Could you check a few things on this model? Use its own coordinates, in mm. Face numbers are marked on the shaded views. A direction names the side the tool comes from. Coordinates: 2 decimals unless noted, no trailing zeros. Loops run counter-clockwise (first coordinate to the right, second up) from the corner with the lowest first, then second, coordinate; pieces in that order, holes last. Notation, with made-up numbers: (8, -23.75) - (14, -23.75) arc R11 cw to (14, -7.75) - close; hole circle Ø9 at (-31.5, -8). An arc over 180 degrees is marked (long way). Use CSV: the item, a comma, the result in double quotes.
from build123d import *

# Parameters (mm, degrees)
EXTRUDE_THIN1_DEPTH      = 10
M4_CLEARANCE_HOLE1_D     = 4.5
M4_CLEARANCE_HOLE1_DEPTH = 124.5
M4_CLEARANCE_HOLE1_TIP   = 1.351936393
FILLET1_R                = 2


with BuildPart() as part:
    # Sketch1 → Extrude-Thin1 (new body)
    with BuildSketch(Plane.XY):
        with BuildLine():
            Line((41.968719423, 0), (31.937438845, 0))
            ThreePointArc((31.937438845, 0), (15.968719423, 15), (0, 0))
            Line((0, 0), (-10.031280577, 0))
            Line((-10.031280577, 0), (-10.031280577, 2))
            Line((-10.031280577, 2), (-1.779519927, 2))
            ThreePointArc((-1.779519927, 2), (15.968719423, 17), (33.716958772, 2))
            Line((33.716958772, 2), (41.968719423, 2))
            Line((41.968719423, 2), (41.968719423, 0))
        make_face()
    extrude(amount=-EXTRUDE_THIN1_DEPTH)

    # M4 Clearance Hole1
    with Locations(Plane(origin=(0, 2, 0), x_dir=(1, 0, 0), z_dir=(0, 1, 0))):
        with Locations((-6.031280577, 5), (37.968719423, 5)):
            Hole(M4_CLEARANCE_HOLE1_D / 2, depth=M4_CLEARANCE_HOLE1_DEPTH)
            with Locations((0, 0, -(M4_CLEARANCE_HOLE1_DEPTH + M4_CLEARANCE_HOLE1_TIP / 2))):  # 118° drill point
                Cone(0, M4_CLEARANCE_HOLE1_D / 2, M4_CLEARANCE_HOLE1_TIP, mode=Mode.SUBTRACT)

    # Fillet1
    fillet1_edges = [part.edges().sort_by_distance(p)[0] for p in [
        (-10.031280577, 1, -10),
        (41.968719423, 1, -10),
        (-10.031280577, 1, 0),
        (41.968719423, 1, 0),
    ]]
    fillet(fillet1_edges, radius=FILLET1_R)


solid = part.part
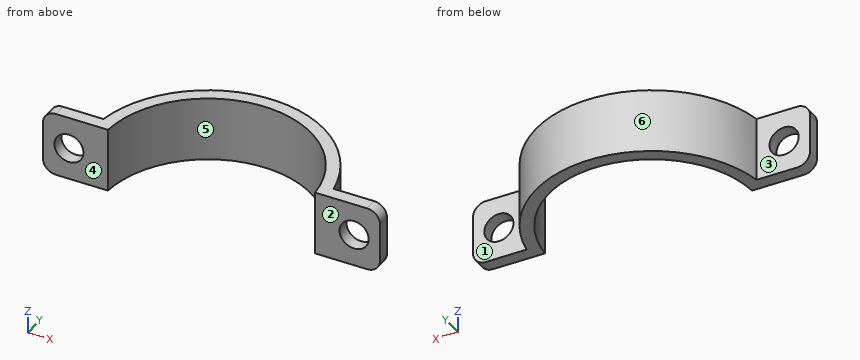
(1) Suppose I cut it at C-C (z = -1.25). Write out the boundary of the cut face in (x, y), plus the area to 3 significant figures.
Computed:
outline,"(-9.89, 0) - (0, 0) arc R16 cw to (31.94, 0) - (41.82, 0) - (41.82, 2) - (33.72, 2) arc R18 ccw to (-1.78, 2) - (-9.89, 2) - close"
area,"135 mm²"
(2) Please list where these lines run through material, in increasing order: line 1 (X direction, y = 0.75, z = -6); line 2 (X direction, y = 7.25, z = -9.5); line 3 (Y direction, x = 35.5, z = -9).
Computed:
line 1,"x = -10.03 to -8.05, -4.02 to 0.06, 31.87 to 35.95, 39.98 to 41.97"
line 2,"x = -0.03 to 2.26, 29.68 to 31.97"
line 3,"y = 0 to 2"
(3) Suppose I cut it at A-A (z = -5). Write out the boundary of the cut face in (x, y), plus the area to 3 significant figures.
Computed:
outline,"(-10.03, 0) - (-8.28, 0) - (-8.28, 2) - (-10.03, 2) - close; (-3.78, 0) - (0, 0) arc R16 cw to (31.94, 0) - (35.72, 0) - (35.72, 2) - (33.72, 2) arc R18 ccw to (-1.78, 2) - (-3.78, 2) - close; (40.22, 0) - (41.97, 0) - (41.97, 2) - (40.22, 2) - close"
area,"117 mm²"
(4) Will these pins go through, and if not, where does the flat tip stop? pin 1 (3 mm diameter, centred on x = 27.5, z = -1.5, fed in from +Y); pin 2 (2 mm diameter, centred on x = 29, y = 6, fed in from -Z); pin 3 (2 mm diameter, centred on y = 5, z = -2.5, fed in from -X); pin 4 (3 mm diameter, centred on x = 17.5, y = 14.5, fed in from -Z).
Computed:
pin 1,"stops at y = 13.95"
pin 2,"passes through"
pin 3,"stops at x = -1.32"
pin 4,"stops at z = -10"
(5) Suppose I cut it at B-B (y = 5). Write out the boundary of the cut face in (x, z).
Computed:
outline,"(-1, -10) - (1.14, -10) - (1.14, 0) - (-1, 0) - close; (30.8, -10) - (32.94, -10) - (32.94, 0) - (30.8, 0) - close"
(6) Which directions (+Z, -Z, +X, -X, +Y, -Y) give clear straight access to the entire face, cutting with the end or side of a thin tool? Please do the marked faces 1, 2 and 3.
Computed:
face 1,"+Z, -Z, +X, +Y"
face 2,"+Z, -Z, +X, -X, -Y"
face 3,"+Z, -Z, -X, +Y"
(7) Suppose I cut it at D-D (x = 23.5). Write out the boundary of the cut face in (y, z).
Computed:
outline,"(13.12, -10) - (15.35, -10) - (15.35, 0) - (13.12, 0) - close"
(8) Thinking about a two-plate mould opening in X: for the marked faces 4, 5 and 6, which applies, +X half, -X half, draft (parallel to the pull), parting line (faces both ways), or undercut?
Computed:
face 4,"draft"
face 5,"undercut"
face 6,"parting line"
